from build123d import *


with BuildPart() as part:
    # Sketch1 → Boss-Revolve (revolve)
    with BuildSketch(Plane.XY, mode=Mode.PRIVATE) as boss_revolve_sk:
        with BuildLine():
            Line((0, 0), (5.292893219, 0))
            Line((5.292893219, 0), (6, -0.707106781))
            Line((6, -0.707106781), (6, -6))
            Line((6, -6), (5, -6))
            Line((5, -6), (4.5, -5.5))
            Line((4.5, -5.5), (4, -5.5))
            ThreePointArc((4, -5.5), (3.646446609, -5.646446609), (3.5, -6))
            Line((3.5, -6), (3.5, -6.5))
            Line((3.5, -6.5), (4, -7))
            Line((4, -7), (4, -15.292893219))
            Line((4, -15.292893219), (3.292893219, -16))
            Line((3.292893219, -16), (0, -16))
            Line((0, -16), (0, 0))
        make_face()
    revolve(boss_revolve_sk.sketch.rotate(Axis((0, 42.170539173, 0), (0, -1, 0)), 180), axis=Axis((0, 42.170539173, 0), (0, -1, 0)))


solid = part.part
Geometry: final body of the model. Coordinates: model frame, mm. A direction names the side the tool comes from. Round coordinates to 2 decimals unless told otherwise and drop trailing zeros. Order: outer loops, then holes, each group sorted by start corner. A loop starts at its lowest first (then second) coordinate and runs counter-clockwise, first axis right, second up. Notation, with made-up numbers: (14.25, 82) -> (36.25, 82) arc R22 cw to (36.25, 105) -> close; hole circle Ø6 at (63.25, -11). An arc over 180 degrees is marked (long way). Put each result on its own line as item: value. Start each with the question number.
Q1. Reachability of faces 1 (the cylindrical face through (-3.233, -6.254, 1.341)), 2 (the cylindrical face through (0.867, -11.204, 3.905)), 3 (the flat face through (0, -16, 0)) from +Z, -Z, +X, -X, +Y, -Y: full face, straight path, thin tool, end or side. Return the list, or none.
Q2. Pull-direction query (Z, two-part tool) for faces 4 (the flat face through (3, -5.5, 3)), 5 (the cylindrical face through (-5.723, -3.391, -1.802)), 6 (the flat face through (4, -6, -4)); classes: +Z half, -Z half, draft (parallel to the pull), parting line (faces both ways), or undercut.
Q3. First-contact query: pin 1 (5 mm diameter, centred on y = -12.5, z = 2.5, fed in from +X); pin 2 (2 mm diameter, centred on x = -1, y = -4, fed in from +Z); pin 3 (5 mm diameter, centred on x = -1, y = -10.5, fed in from -Z); pin 4 (5 mm diameter, centred on y = -11, z = 2.5, fed in from -X). Flat tips, straight axial feed; report the tip coordinate or a pass-through.
Q4. Section B-B on x = 0. Return the cut outline in (y, z).
Q5. Section A-A on z = 0. Return the cut outline in (x, y), and give its area (3 significant figures).
Q6. Line query: probe 1 along Z at (x, y) = (0.25, -3.25); probe 2 along Y at (x, z) = (-4.25, -1); probe 3 along Y at (x, z) = (5, 1.5). Output: solid intervals per line, ascending.
Q7. Section C-C on y = -14. Return the cut outline in (x, z).
Ans:
1. face 1: none
1. face 2: -Y
1. face 3: +Z, -Z, +X, -X, -Y
2. face 4: undercut
2. face 5: parting line
2. face 6: draft
3. pin 1: stops at x = 4
3. pin 2: stops at z = 6
3. pin 3: stops at z = -4
3. pin 4: stops at x = -4
4. outline: (-16, -3.29) -> (-15.29, -4) -> (-7, -4) -> (-6.5, -3.5) -> (-6, -3.5) arc R0.5 cw to (-5.5, -4) -> (-5.5, -4.5) -> (-6, -5) -> (-6, -6) -> (-0.71, -6) -> (0, -5.29) -> (0, 5.29) -> (-0.71, 6) -> (-6, 6) -> (-6, 5) -> (-5.5, 4.5) -> (-5.5, 4) arc R0.5 cw to (-6, 3.5) -> (-6.5, 3.5) -> (-7, 4) -> (-15.29, 4) -> (-16, 3.29) -> close
5. outline: (-6, -6) -> (-5, -6) -> (-4.5, -5.5) -> (-4, -5.5) arc R0.5 cw to (-3.5, -6) -> (-3.5, -6.5) -> (-4, -7) -> (-4, -15.29) -> (-3.29, -16) -> (3.29, -16) -> (4, -15.29) -> (4, -7) -> (3.5, -6.5) -> (3.5, -6) arc R0.5 cw to (4, -5.5) -> (4.5, -5.5) -> (5, -6) -> (6, -6) -> (6, -0.71) -> (5.29, 0) -> (-5.29, 0) -> (-6, -0.71) -> close
5. area: 149 mm2
6. probe 1: z = -5.99 to 5.99
6. probe 2: y = -5.5 to 0
6. probe 3: y = -6 to 0
7. outline: circle Ø8 at (0, 0)
